Geometry: final body of the model. Coordinates: model frame, mm. A direction names the side the tool comes from. Round coordinates to 2 decimals unless told otherwise and drop trailing zeros. Write each loop counter-clockwise with the first axis right and the second up, starting at its lowest first coordinate (ties: lowest second). Pieces come first, ordered by that corner, then holes. Notation, with made-up numbers: (3.5, 61) -> (60.5, 61) arc R19 ccw to (60.5, 94) -> close; hole circle Ø10 at (30.5, 76.5). An arc over 180 degrees is marked (long way). Use one line per item in the form item = value. Start each with the question number.
1. Line query: L1, parallel to Y at x = 48.5, z = 113.5; L2, parallel to Y at x = 49.5, z = 6.5; L3, parallel to X at y = 12, z = -213.5. Output: solid intervals per line, ascending.
2. Pin query (flat end, axial travel): pin 1 Ø10 at (y, z) = (23.5, 223.5) entering from +X. Return the tip coordinate at first contact, or that it passes through.
3. Draft query along Y for faces 1 (the face through (31.102, 54.316, 8.307)), 2 (the face through (0, 1, 4)), 3 (the face through (26, -63, 4)). Return one class per face: pulls with the +Y half, pulls with the -Y half, needs draft (parallel to the pull), parting line crosses it, or undercut.
4. Cut plane C-C, the plane y = 32. Return the cut outline in (x, z), plus the area to 3 significant figures.
5. Cut plane B-B, the plane x = 39. Return the cut outline in (y, z).
6. Reachability of faces 4 (the face through (31.59, -54.35, 8.31)), 5 (the face through (4.784, 0.294, 302.954)) from +Z, -Z, +X, -X, +Y, -Y: full face, straight path, thin tool, end or side. Return the list, or none.
7. Cut plane A-A, the plane z = 129.5. Return the cut outline in (x, y).
```python
from build123d import *

# Parameters (mm, degrees)
BOSS_EXTRUDE1_DEPTH = 306.5
CUT_EXTRUDE1_DEPTH  = 613


with BuildPart() as part:
    # Sketch1 → Boss-Extrude1 (new, symmetric)
    with BuildSketch(Plane.XY):
        with BuildLine():
            Line((0, 63), (0, -63))
            Line((0, -63), (53, -63))
            Line((53, -63), (53, -60.015930389))
            ThreePointArc((53, -60.015930389), (51.788680261, -56.944353898), (48.806852383, -55.526404621))
            Line((48.806852383, -55.526404621), (13.886295235, -53.139636681))
            ThreePointArc((13.886295235, -53.139636681), (7.922639477, -50.303738128), (5.5, -44.160585147))
            Line((5.5, -44.160585147), (5.5, 44.160585147))
            ThreePointArc((5.5, 44.160585147), (7.922639477, 50.303738128), (13.886295235, 53.139636681))
            Line((13.886295235, 53.139636681), (48.806852383, 55.526404621))
            ThreePointArc((48.806852383, 55.526404621), (51.788680261, 56.944353898), (53, 60.015930389))
            Line((53, 60.015930389), (53, 63))
            Line((53, 63), (0, 63))
        make_face()
    extrude(amount=BOSS_EXTRUDE1_DEPTH, both=True)

    # Sketch2 → Cut-Extrude1 (cut)
    with BuildSketch(Plane(origin=(0, 63, 0), x_dir=(1, 0, 0), z_dir=(0, 1, 0))):
        Polygon((0, -306.5), (53, -267.210441025), (53, -306.5), align=None)
        Polygon((0, 306.5), (53, 235.005178647), (53, 306.5), align=None)
    extrude(amount=-CUT_EXTRUDE1_DEPTH, mode=Mode.SUBTRACT)


solid = part.part
```
Outcome:
q1.L1 = -63 to -55.51, 55.51 to 63
q1.L2 = -63 to -55.63, 55.63 to 63
q1.L3 = 0 to 5.5
q2.pin_1 = 5.5
q3.face_1 = undercut
q3.face_2 = needs draft
q3.face_3 = pulls with the -Y half
q4.outline = (0, -306.5) -> (5.5, -299.08) -> (5.5, 302.42) -> (0, 306.5) -> close
q4.area = 3,340 mm^2
q5.outline = (-63, -253.89) -> (-54.86, -253.89) -> (-54.86, 277.59) -> (-63, 277.59) -> close; (54.86, -253.89) -> (63, -253.89) -> (63, 277.59) -> (54.86, 277.59) -> close
q6.face_4 = +Z, -Z, +X
q6.face_5 = +Z, +X, +Y, -Y
q7.outline = (0, -63) -> (53, -63) -> (53, -60.02) arc R4.5 ccw to (48.81, -55.53) -> (13.89, -53.14) arc R9 cw to (5.5, -44.16) -> (5.5, 44.16) arc R9 cw to (13.89, 53.14) -> (48.81, 55.53) arc R4.5 ccw to (53, 60.02) -> (53, 63) -> (0, 63) -> close
